from build123d import *

# Parameters (mm, degrees)
BASE_BODY_DEPTH         = 46
SIDE_BLOCK_SKETCH_W     = 10
SIDE_BLOCK_SKETCH_H     = 25
SIDE_BLOCK_DEPTH        = 23
FRONT_BLOCK_DEPTH       = 23
LUG_DEPTH               = 10
LUG_EXTENSION_SKETCH_R  = 5
LUG_EXTENSION_DEPTH     = 10
PIN_HOLE_SKETCH_R       = 5
LUG_PIN_HOLE_DEPTH      = 10
SLOT_SKETCH_W           = 20
SLOT_SKETCH_H           = 19.323161221
SLOT_CUT_DEPTH          = 19
ANGLED_RELIEF_CUT_DEPTH = 81


with BuildPart() as part:
    # Base Profile Sketch → Base Body (new body)
    with BuildSketch(Plane(origin=(0, 0, 0), x_dir=(0, 0, -1), z_dir=(1, 0, 0))):
        Polygon((50.202309924, 0), (-50.202309924, 0), (-50.202309924, -15), (-20.202309924, -15), (-20.202309924, -30), (20.202309924, -30), (20.202309924, -15), (50.202309924, -15), align=None)
    extrude(amount=BASE_BODY_DEPTH)

    # Side Block Sketch → Side Block (add, symmetric)
    with BuildSketch(Plane(origin=(23, 0, 0), x_dir=(0, 0, -1), z_dir=(1, 0, 0))):
        with Locations((-10.202309924, 12.5)):
            Rectangle(SIDE_BLOCK_SKETCH_W, SIDE_BLOCK_SKETCH_H)
    extrude(amount=SIDE_BLOCK_DEPTH, both=True)

    # Front Block Sketch → Front Block (add, symmetric)
    with BuildSketch(Plane(origin=(23, 0, 0), x_dir=(0, 0, -1), z_dir=(1, 0, 0))):
        Polygon((-5.202309924, 13.015188061), (26.202309924, 0), (-5.202309924, 0), (-5.202309924, 13), align=None)
    extrude(amount=FRONT_BLOCK_DEPTH, both=True)

    # Lug Sketch → Lug (add)
    with BuildSketch(Plane(origin=(0, 0, 5.202309924), x_dir=(-1, 0, 0), z_dir=(0, 0, -1))):
        with BuildLine():
            ThreePointArc((-33, 25), (-23, 35), (-13, 25))
            Line((-13, 25), (0, 25))
            ThreePointArc((0, 25), (-23, 48), (-46, 25))
            Line((-46, 25), (-33, 25))
        make_face()
    extrude(amount=-LUG_DEPTH)

    # Lug Extension Sketch → Lug Extension (add)
    with BuildSketch(Plane(origin=(0, 0, 5.202309924), x_dir=(-1, 0, 0), z_dir=(0, 0, -1))):
        with Locations((-23, 25)):
            Circle(LUG_EXTENSION_SKETCH_R)
        with BuildLine():
            Line((-13, 25), (-33, 25))
            ThreePointArc((-33, 25), (-23, 35), (-13, 25))
        make_face()
        with BuildLine():
            ThreePointArc((-28, 25), (-23, 20), (-18, 25))
            Line((-18, 25), (-28, 25))
        make_face()
        with BuildLine():
            Line((-28, 25), (-18, 25))
            ThreePointArc((-18, 25), (-23, 30), (-28, 25))
        make_face()
    extrude(amount=-LUG_EXTENSION_DEPTH)

    # Pin Hole Sketch → Lug Pin Hole (cut)
    with BuildSketch(Plane(origin=(0, 0, 5.202309924), x_dir=(-1, 0, 0), z_dir=(0, 0, -1))):
        with Locations((-23, 25)):
            Circle(PIN_HOLE_SKETCH_R)
    extrude(amount=-LUG_PIN_HOLE_DEPTH, mode=Mode.SUBTRACT)

    # Slot Sketch → Slot Cut (cut)
    with BuildSketch(Plane(origin=(0, 0, 0), x_dir=(1, 0, 0), z_dir=(0, 1, 0))):
        with Locations((23, 50.202309924)):
            Rectangle(SLOT_SKETCH_W, SLOT_SKETCH_H)
    extrude(amount=-SLOT_CUT_DEPTH, mode=Mode.SUBTRACT)

    # Angled Cut Sketch → Angled Relief Cut (cut)
    with BuildSketch(Plane(origin=(0, 0, -20.202309924), x_dir=(-1, 0, 0), z_dir=(0, 0, -1))):
        Polygon((-23, -15), (-32.5, -15), (-32.5, -32.214795119), (-13.5, -32.214795119), (-13.5, -15), align=None)
    extrude(amount=-ANGLED_RELIEF_CUT_DEPTH, mode=Mode.SUBTRACT)


solid = part.part
For this review, take the finished solid that the model builds, in its own axes (mm). A direction names the side the tool comes from. Give positions to 0.01 mm unless a question says otherwise; leave off trailing zeros. Order: outer loops, then holes, each group sorted by start corner. A loop starts at its lowest first (then second) coordinate and runs counter-clockwise, first axis right, second up. Notation, with made-up numbers: M 48,25 L 88,25 A19 cw 88,56 Z; hole C -30,46 d4. An arc over 180 degrees is marked long. Answer in a Markdown table with one row per item. Add a question column.
(1) Consider section B-B on x = 23. State the section outline as (y, z) points.
(2) For faces 1 (the face through (23, 0, -36)), 2 (the face through (23, 0, 32)), 3 (the face through (7, -23, -20.202)), 4 (the face through (7, -22, 20.202)), 5 (the face through (23, -7, -40.541)), list the 3-axis set-ups (+Z, -Z, +X, -X, +Y, -Y) from which the entire face can be reached by the end or side of a thin tool; tool diameter is ignored.
(3) Consider section D-D on z = -11. State the section outline as (x, y) points, and give its area (3 significant figures).
(4) Consider section A-A on z = 10.5. State the section outline as (x, y) points, and give its area (3 significant figures).
(5) For pin 1 (1.5 mm diameter, centred on x = 15, z = -33.5, fed in from +Y); pin 2 (23 mm diameter, centred on x = 34, y = 20, fed in from +Z); pin 3 (15 mm diameter, centred on x = 40, y = -23, fed in from -Z), all flat-tipped, find the tip position at first contact; note any pin that passes through.
(6) Mouldability with a two-part tool opening along X and no side actions: class faces 6 (the face through (46, -8, -1)), 7 (the face through (23, 19, 15.202)), 8 (the face through (13.5, -23, 0)), 9 (the face through (22.494, 47.994, 10.132)) as +X half, -X half, draft (parallel to the pull), parting line (faces both ways), or undercut.
(7) Consider section C-C on y = -12.5. State the section outline as (x, z) points.
(8) Wall thickness on probe 1 along Y at (x, z) = (23, 12.5); probe 2 along Z at (x, y) = (31, 43); probe 3 along Y at (x, z) = (29, -36): over which ranges is each line inside the solid? List them lowest first. Write a range as [from, to].
Evaluation:
| question | item | result |
|---|---|---|
| 1 | outline | M -15,-40.54 L 0,-40.54 L 0,-26.2 L 13.02,5.2 L 20,5.2 L 20,15.2 L 0,15.2 L 0,50.2 L -15,50.2 Z; M 30,5.2 L 48,5.2 L 48,15.2 L 30,15.2 Z |
| 2 | face 1 | -Z, +X, -X, +Y |
| 2 | face 2 | +Z, +X, -X, +Y |
| 2 | face 3 | -Z, +X, -X, -Y |
| 2 | face 4 | +Z, +X, -X, -Y |
| 2 | face 5 | -Z, +Y, -Y |
| 3 | outline | M 0,-30 L 13.5,-30 L 13.5,-15 L 32.5,-15 L 32.5,-30 L 46,-30 L 46,6.3 L 0,6.3 Z |
| 3 | area | 1,380 mm^2 |
| 4 | outline | M 0,-30 L 13.5,-30 L 13.5,-15 L 32.5,-15 L 32.5,-30 L 46,-30 L 46,25 A23 ccw 0,25 Z; hole C 23,25 d10 |
| 4 | area | 3,000 mm^2 |
| 5 | pin 1 | stops at y = 0 |
| 5 | pin 2 | stops at z = 15.2 |
| 5 | pin 3 | stops at z = -20.2 |
| 6 | face 6 | +X half |
| 6 | face 7 | draft |
| 6 | face 8 | undercut |
| 6 | face 9 | parting line |
| 7 | outline | M 0,-50.2 L 13,-50.2 L 13,-40.54 L 33,-40.54 L 33,-50.2 L 46,-50.2 L 46,50.2 L 0,50.2 Z |
| 8 | probe 1 | y = [-15, 20], [30, 48] |
| 8 | probe 2 | z = [5.2, 15.2] |
| 8 | probe 3 | y = [-15, 0] |
